from build123d import *

# Parameters (mm, degrees)
SKETCH2_W           = 150
SKETCH2_H           = 25
BOSS_EXTRUDE1_DEPTH = 15
SKETCH3_R           = 30
BOSS_EXTRUDE2_DEPTH = 30
SKETCH4_R           = 5.5
CUT_EXTRUDE1_DEPTH  = 30
BOSS_EXTRUDE3_START = -120
SKETCH5_R           = 30
BOSS_EXTRUDE3_DEPTH = 120


with BuildPart() as part:
    # Sketch2 → Boss-Extrude1 (new, symmetric)
    with BuildSketch(Plane.XY):
        Rectangle(SKETCH2_W, SKETCH2_H)
    extrude(amount=BOSS_EXTRUDE1_DEPTH, both=True)

    # Sketch3 → Boss-Extrude2 (add)
    with BuildSketch(Plane.XY.offset(15)):
        with BuildLine():
            Line((-15, 87.5), (-15, 0))
            Line((-15, 0), (75, 0))
            Line((75, 0), (75, 87.5))
            ThreePointArc((75, 87.5), (30, 132.5), (-15, 87.5))
        make_face()
        with Locations((30, 87.5)):
            Circle(SKETCH3_R, mode=Mode.SUBTRACT)
    extrude(amount=-BOSS_EXTRUDE2_DEPTH)

    # Sketch4 → Cut-Extrude1 (cut)
    with BuildSketch(Plane(origin=(0, 12.5, 0), x_dir=(1, 0, 0), z_dir=(0, 1, 0))):
        with Locations(Location((-60, 0, 0), (0, 0, 270))):
            Circle(SKETCH4_R)
        with Locations(Location((-40, 0, 0), (0, 0, 270))):
            Circle(SKETCH4_R)
    extrude(amount=-CUT_EXTRUDE1_DEPTH, mode=Mode.SUBTRACT)

    # Sketch5 → Boss-Extrude3 (add)
    with BuildSketch(Plane(origin=(0, 0, -15), x_dir=(-1, 0, 0), z_dir=(0, 0, -1)).offset(BOSS_EXTRUDE3_START)):
        with Locations((-30, 87.5)):
            Circle(SKETCH5_R)
    extrude(amount=BOSS_EXTRUDE3_DEPTH)


solid = part.part
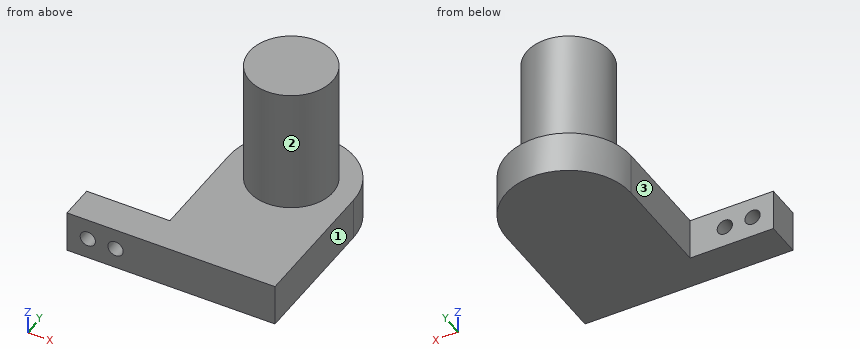
Input: part model. Units: mm. Frame: model coordinates. Face numbers are marked on the shaded views. A direction names the side the tool comes from. Coordinates: 2 decimals unless noted, no trailing zeros. Loops run counter-clockwise (first coordinate to the right, second up) from the corner with the lowest first, then second, coordinate; pieces in that order, holes last. Notation, with made-up numbers: (-31.75, 1) -> (-16.75, 1) arc R10 ccw to (-16.75, 9) -> close; hole circle Ø6 at (29.5, 62.5). An arc over 180 degrees is marked (long way). Write item = value, one per line. Start each with the question number.
Item 1: Cut plane A-A, the plane x = -40. Return loops of the section in (y, z), plus the area to 3 significant figures.
Item 2: First-contact query: P1, Ø8, axis at y = 30, z = 18.5, coming from the +X side; P2, Ø17.5, axis at x = -60, z = 0, coming from the +Y side; P3, Ø1, axis at y = 64, z = 28.5, coming from the -X side; P4, Ø4, axis at y = 61.5, z = 48, coming from the +X side. Flat tips, straight axial feed; report the tip coordinate or a pass-through.
Item 3: Cut plane C-C, the plane x = 30. Return loops of the section in (y, z).
Item 4: Cut plane B-B, the plane z = 0. Return loops of the section in (x, y), plus the area to 3 significant figures.
Item 5: Material intervals for line 1 (X direction, y = -2.25, z = 0); line 2 (X direction, y = 26.5, z = -2); line 3 (Z direction, x = 16, y = 57), sorted ascending.
Item 6: Cut plane D-D, the plane y = 69.5. Return loops of the section in (x, z), plus the area to 3 significant figures.
Item 7: Reachability of the marked faces 1, 2 and 3 from +Z, -Z, +X, -X, +Y, -Y: full face, straight path, thin tool, end or side. Return the list, or none.
Ans:
q1.outline = (-12.5, -15) -> (12.5, -15) -> (12.5, -5.5) -> (-12.5, -5.5) -> close; (-12.5, 5.5) -> (12.5, 5.5) -> (12.5, 15) -> (-12.5, 15) -> close
q1.area = 475 mm²
q2.P1 = 75
q2.P2 = 12.5
q2.P3 = 10.74
q2.P4 = 48
q3.outline = (-12.5, -15) -> (132.5, -15) -> (132.5, 15) -> (117.5, 15) -> (117.5, 105) -> (57.5, 105) -> (57.5, 15) -> (-12.5, 15) -> close
q4.outline = (-75, -12.5) -> (-65.5, -12.5) -> (-65.5, 12.5) -> (-75, 12.5) -> close; (-54.5, -12.5) -> (-45.5, -12.5) -> (-45.5, 12.5) -> (-54.5, 12.5) -> close; (-34.5, -12.5) -> (75, -12.5) -> (75, 87.5) arc R45 ccw to (-15, 87.5) -> (-15, 12.5) -> (-34.5, 12.5) -> close
q4.area = 13,100 mm²
q5.line_1 = -75 to -65.5, -54.5 to -45.5, -34.5 to 75
q5.line_2 = -15 to 75
q5.line_3 = -15 to 15
q6.outline = (-15, -15) -> (75, -15) -> (75, 15) -> (54, 15) -> (54, 105) -> (6, 105) -> (6, 15) -> (-15, 15) -> close
q6.area = 7,020 mm²
q7.face_1 = +Z, -Z, +X, +Y, -Y
q7.face_2 = +Z
q7.face_3 = +Z, -Z, -X, +Y
